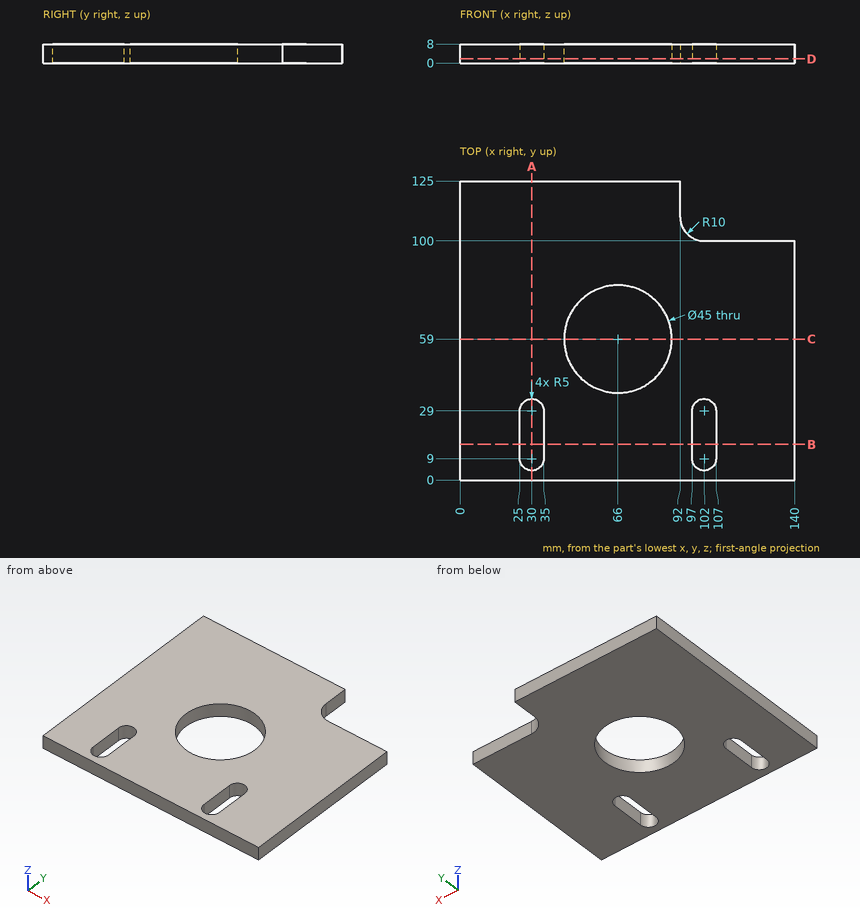
The figure shows three views and two pictorial views of one solid part (mm, origin at its lowest corner). Answer the questions. Coordinates: 2 decimals unless noted, no trailing zeros. Order: outer loops, then holes, each group sorted by start corner. A loop starts at its lowest first (then second) coordinate and runs counter-clockwise, first axis right, second up. Notation, with made-up numbers: (-30, -12.5) - (15, -12.5) arc R18 ccw to (15, 12.5) - close; hole circle Ø8 at (54, 77). An arc over 180 degrees is marked (long way). Answer as a JSON object with one key per item and string values.
1. Consider line 1 (X direction, y = 17, z = 4.25); line 2 (Y direction, x = 66, z = 6.5); line 3 (X direction, y = 7.5, z = 1.25). Determine where each line is inside the solid, lowest interval first.
Output values:
{"line 1": "x = 0 to 25, 35 to 97, 107 to 140", "line 2": "y = 0 to 36.5, 81.5 to 125", "line 3": "x = 0 to 25.23, 34.77 to 97.23, 106.77 to 140"}
2. Find section B-B on y = 15. Determine the outline of the cut face in (x, z), plus the area to 3 significant figures.
Output values:
{"outline": "(0, 0) - (25, 0) - (25, 8) - (0, 8) - close; (35, 0) - (97, 0) - (97, 8) - (35, 8) - close; (107, 0) - (140, 0) - (140, 8) - (107, 8) - close", "area": "960 mm²"}
3. Find section C-C on y = 59. Determine the outline of the cut face in (x, z).
Output values:
{"outline": "(0, 0) - (43.5, 0) - (43.5, 8) - (0, 8) - close; (88.5, 0) - (140, 0) - (140, 8) - (88.5, 8) - close"}
4. Find section D-D on z = 1.75. Determine the outline of the cut face in (x, y).
Output values:
{"outline": "(0, 0) - (140, 0) - (140, 100) - (102, 100) arc R10 cw to (92, 110) - (92, 125) - (0, 125) - close; hole (25, 9) arc R5 ccw to (35, 9) - (35, 29) arc R5 ccw to (25, 29) - close; hole circle Ø45 at (66, 59); hole (97, 9) arc R5 ccw to (107, 9) - (107, 29) arc R5 ccw to (97, 29) - close"}
5. Find section A-A on x = 30. Determine the outline of the cut face in (y, z), plus the area to 3 significant figures.
Output values:
{"outline": "(0, 0) - (4, 0) - (4, 8) - (0, 8) - close; (34, 0) - (125, 0) - (125, 8) - (34, 8) - close", "area": "760 mm²"}
6. Each of these flat-tipped pins is pushed along its axis until it touches: P1, Ø4, axis at x = 116, z = 2, coming from the +Y side; P2, Ø2.5, axis at y = 118.5, z = 3, coming from the +X side. Where does it stop, or does it pass through?
Output values:
{"P1": "stops at y = 100", "P2": "stops at x = 92"}
